```python
from build123d import *

# Parameters (mm, degrees)
SKETCH1_R                 = 6.5
BOSS_EXTRUDE1_DEPTH       = 0.5
SKETCH3_R                 = 8.5
BOSS_EXTRUDE3_DEPTH       = 6
CHAMFER2_SIZE             = 0.5
SKETCH4_W                 = 4.01520781
SKETCH4_H                 = 18.659876277
SKETCH4_W_2               = 10.097066699
SKETCH4_H_2               = 2.598075642
SKETCH4_W_3               = 5.358269855
SKETCH4_H_3               = 23.485379118
SKETCH4_W_4               = 10.284722044
SKETCH4_H_4               = 2.952358684
CUT_EXTRUDE3_DEPTH        = 14.435028843
M8X1_0_TAPPED_HOLE1_D     = 7
M8X1_0_TAPPED_HOLE1_DEPTH = 19
M8X1_0_TAPPED_HOLE1_TIP   = 2.103012167
SKETCH7_W                 = 1.25
SKETCH7_H                 = 9.899494937
CHAMFER3_SIZE             = 0.5
CIRPATTERN1_COUNT         = 2
CIRPATTERN1_ANGLE         = 90


with BuildPart() as part:
    # Sketch1 → Boss-Extrude1 (new body)
    with BuildSketch(Plane(origin=(0, 0, 0), x_dir=(1, 0, 0), z_dir=(0, 1, 0))):
        with Locations(Location((0, 0, 0), (0, 0, 270))):
            Circle(SKETCH1_R)
    extrude(amount=BOSS_EXTRUDE1_DEPTH)

    # Sketch3 → Boss-Extrude3 (add)
    with BuildSketch(Plane.XZ):
        with Locations(Location((0, 0, 0), (0, 0, 270))):
            Circle(SKETCH3_R)
    extrude(amount=BOSS_EXTRUDE3_DEPTH)

    # Chamfer2
    chamfer2_edges = [part.edges().sort_by_distance(p)[0] for p in [
        (0, 0, 8.5),
        (0, -6, 8.5),
    ]]
    chamfer(chamfer2_edges, length=CHAMFER2_SIZE)

    # Sketch4 → Cut-Extrude3 (cut, through all)
    with BuildSketch(Plane(origin=(0, 0, 0), x_dir=(1, 0, 0), z_dir=(0, 1, 0))):
        with Locations((-9.007603905, 1.516224116)):
            Rectangle(SKETCH4_W, SKETCH4_H)
        with Locations((0.059047173, 8.299037821)):
            Rectangle(SKETCH4_W_2, SKETCH4_H_2)
        with Locations((9.679134928, -0.60539293)):
            Rectangle(SKETCH4_W_3, SKETCH4_H_3)
        with Locations((-0.142361022, -8.476179342)):
            Rectangle(SKETCH4_W_4, SKETCH4_H_4)
    extrude(amount=-CUT_EXTRUDE3_DEPTH, mode=Mode.SUBTRACT)

    # M8x1.0 Tapped Hole1
    with Locations(Plane(origin=(0, 0.5, 0), x_dir=(-1, 0, 0), z_dir=(0, 1, 0))):
        with Locations((0, 0)):
            Hole(M8X1_0_TAPPED_HOLE1_D / 2, depth=M8X1_0_TAPPED_HOLE1_DEPTH)
            with Locations((0, 0, -(M8X1_0_TAPPED_HOLE1_DEPTH + M8X1_0_TAPPED_HOLE1_TIP / 2))):  # 118° drill point
                Cone(0, M8X1_0_TAPPED_HOLE1_D / 2, M8X1_0_TAPPED_HOLE1_TIP, mode=Mode.SUBTRACT)

    # Sketch7 → M3 Tapped Hole1 (revolve, cut)
    with BuildSketch(Plane(origin=(0, -3, 0), x_dir=(0.7071067811865488, 0, 0.7071067811865464), z_dir=(0, 1, 0))):
        with Locations((0.625, 4.949747469)):
            Rectangle(SKETCH7_W, SKETCH7_H)
    m3_tapped_hole1 = revolve(axis=Axis((-4.490128061, -3, 4.490128061), (0.7071067811865464, 0, -0.7071067811865487)), mode=Mode.SUBTRACT)

    # Chamfer3
    chamfer3_edges = [part.edges().sort_by_distance(p)[0] for p in [
        (-3.5, -6, 0),
        (-3.5, 0.5, 0),
    ]]
    chamfer(chamfer3_edges, length=CHAMFER3_SIZE)

    # CirPattern1: M3 Tapped Hole1 ×2 about axis
    cirpattern1_axis = Axis((0, 0.5, 0), (0, 1, 0))
    for i in range(1, CIRPATTERN1_COUNT):
        add(m3_tapped_hole1.rotate(cirpattern1_axis, i * CIRPATTERN1_ANGLE / (CIRPATTERN1_COUNT - 1)), mode=Mode.SUBTRACT)


solid = part.part
```
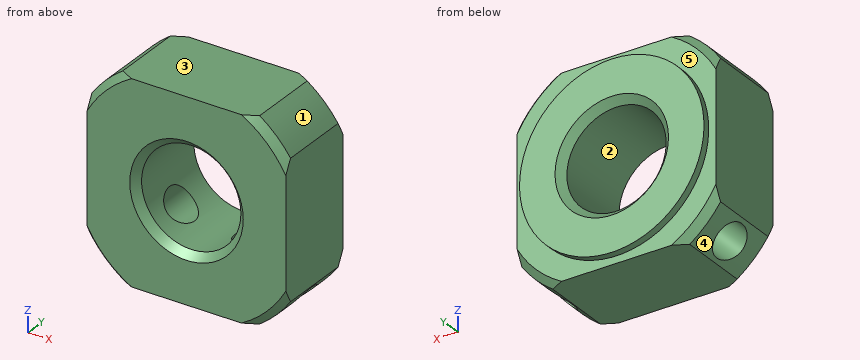
Can you work these out from the model? Positions are in its coordinate system, mm. Face numbers are marked on the shaded views. A direction names the side the tool comes from. Round coordinates to 2 decimals unless told otherwise and drop trailing zeros. Loops run counter-clockwise (first coordinate to the right, second up) from the corner with the lowest first, then second, coordinate; pieces in that order, holes last.
Item 1: Suppose I cut it at A-A, the plane z = 0. Write out the boundary of the cut face in (x, y), then the cut area to 3 significant figures.
Item 2: Which directions (+Z, -Z, +X, -X, +Y, -Y) give clear straight access to the entire face, cutting with the end or side of a thin tool? Please do the marked faces 4 and 5.
Item 3: Please list where these lines run through material, in increasing order: L1, parallel to Z at x = 0, y = -2; L2, parallel to X at y = -0.5, z = 0.25; L3, parallel to Y at x = -6.5, z = -2.25.
Item 4: If we mould it in two halves opening along X, with no side actions, what happens to the marked faces 1, 2 and 3? For each: +X half, -X half, draft (parallel to the pull), parting line (faces both ways), or undercut.
Item 5: Will this pin go through, and if not, where does the flat tip stop? pin 1 Ø6.5 at (x, z) = (0, 0) entering from -Y.
Item 6: Suppose I cut it at C-C, the plane y = -4.75. Write out the boundary of the cut face in (x, z), then the cut area to 3 significant figures.
Item 7: Suppose I cut it at B-B, the plane x = 0. Write out the boundary of the cut face in (y, z).
Reported:
1. outline: (-7, -6) - (-4, -6) - (-3.5, -5.5) - (-3.5, 0) - (-4, 0.5) - (-6.5, 0.5) - (-6.5, 0) - (-7, 0) - close; (3.5, -5.5) - (4, -6) - (7, -6) - (7, 0) - (6.5, 0) - (6.5, 0.5) - (4, 0.5) - (3.5, 0) - close
1. area: 44.5 mm2
2. face 4: -Z, -X, +Y, -Y
2. face 5: +Y
3. L1: z = -7 to -3.5, 3.5 to 7
3. L2: x = -7 to -3.49, 3.49 to 7
3. L3: y = -6 to 0
4. face 1: +X half
4. face 2: undercut
4. face 3: draft
5. pin 1: passes through
6. outline: (-7, -4.82) arc R8.5 ccw to (-4.82, -7) - (4.82, -7) arc R8.5 ccw to (7, -4.82) - (7, 4.82) arc R8.5 ccw to (4.82, 7) - (-4.82, 7) arc R8.5 ccw to (-7, 4.82) - close; hole circle Ø7 at (0, 0)
6. area: 149 mm2
7. outline: (-6, -7) - (0, -7) - (0, -6.5) - (0.5, -6.5) - (0.5, -4) - (0, -3.5) - (-5.5, -3.5) - (-6, -4) - close; (-6, 4) - (-5.5, 3.5) - (0, 3.5) - (0.5, 4) - (0.5, 6.5) - (0, 6.5) - (0, 7) - (-6, 7) - close
